Build history of the part. All positions in model axes, mm. Round coordinates to 2 decimals unless told otherwise and drop trailing zeros. Put each result on its own line as item: value. Start each with the question number.
Item 1: Drill centre lines: probe 1 along Y at (x, z) = (165, -16); probe 2 along Z at (x, y) = (-309.5, 5); probe 3 along Z at (x, y) = (425, -15). Where is each one in solid material? Low to high. Write a range as [from, to].
Item 2: Flat gauge pins, fed straight in: pin 1 Ø3 at (x, y) = (170.5, -19) entering from -Z; pin 2 Ø5 at (x, y) = (254, -0.5) entering from +Z; pin 3 Ø2 at (x, z) = (-299, 18.5) entering from -Y. Where does each tip first touch, or does it go through?
Item 3: Cut at A-A, the plane x = -300. Count the separate pieces of the cut face and the enclosed holes in it, plus the area to 3 significant figures.
```python
from build123d import *

# Parameters (mm, degrees)
SKETCH1_R                 = 3.4
SKETCH1_R_2               = 3
F_40_X_40W_X_R4_5_1_DEPTH = 1200


with BuildPart() as part:
    # Sketch1 → 铝型材 40 X 40W X R4.5(1) (new body)
    with BuildSketch(Plane(origin=(-600, 0, 0), x_dir=(0, 0, -1), z_dir=(1, 0, 0))):
        with BuildLine():
            Line((-5.1, 20), (-5.1, 19.5))
            Line((-5.1, 19.5), (-4.1, 19.5))
            Line((-4.1, 19.5), (-4.1, 17))
            Line((-4.1, 17), (-6.1, 17))
            Line((-6.1, 17), (-6.1, 18))
            Line((-6.1, 18), (-10.3, 18))
            Line((-10.3, 18), (-10.3, 12))
            Line((-10.3, 12), (-6, 7.7))
            Line((-6, 7.7), (6, 7.7))
            Line((6, 7.7), (10.3, 12))
            Line((10.3, 12), (10.3, 18))
            Line((10.3, 18), (6.1, 18))
            Line((6.1, 18), (6.1, 17))
            Line((6.1, 17), (4.1, 17))
            Line((4.1, 17), (4.1, 19.5))
            Line((4.1, 19.5), (5.1, 19.5))
            Line((5.1, 19.5), (5.1, 20))
            Line((5.1, 20), (15.5, 20))
            ThreePointArc((15.5, 20), (18.681980515, 18.681980515), (20, 15.5))
            Line((20, 15.5), (20, 5.1))
            Line((20, 5.1), (19.5, 5.1))
            Line((19.5, 5.1), (19.5, 4.1))
            Line((19.5, 4.1), (17, 4.1))
            Line((17, 4.1), (17, 6.1))
            Line((17, 6.1), (18, 6.1))
            Line((18, 6.1), (18, 10.3))
            Line((18, 10.3), (12, 10.3))
            Line((12, 10.3), (7.7, 6))
            Line((7.7, 6), (7.7, -6))
            Line((7.7, -6), (12, -10.3))
            Line((12, -10.3), (18, -10.3))
            Line((18, -10.3), (18, -6.1))
            Line((18, -6.1), (17, -6.1))
            Line((17, -6.1), (17, -4.1))
            Line((17, -4.1), (19.5, -4.1))
            Line((19.5, -4.1), (19.5, -5.1))
            Line((19.5, -5.1), (20, -5.1))
            Line((20, -5.1), (20, -15.5))
            ThreePointArc((20, -15.5), (18.681980515, -18.681980515), (15.5, -20))
            Line((15.5, -20), (5.1, -20))
            Line((5.1, -20), (5.1, -19.5))
            Line((5.1, -19.5), (4.1, -19.5))
            Line((4.1, -19.5), (4.1, -17))
            Line((4.1, -17), (6.1, -17))
            Line((6.1, -17), (6.1, -18))
            Line((6.1, -18), (10.3, -18))
            Line((10.3, -18), (10.3, -12))
            Line((10.3, -12), (6, -7.7))
            Line((6, -7.7), (-6, -7.7))
            Line((-6, -7.7), (-10.3, -12))
            Line((-10.3, -12), (-10.3, -18))
            Line((-10.3, -18), (-6.1, -18))
            Line((-6.1, -18), (-6.1, -17))
            Line((-6.1, -17), (-4.1, -17))
            Line((-4.1, -17), (-4.1, -19.5))
            Line((-4.1, -19.5), (-5.1, -19.5))
            Line((-5.1, -19.5), (-5.1, -20))
            Line((-5.1, -20), (-15.5, -20))
            ThreePointArc((-15.5, -20), (-18.681980515, -18.681980515), (-20, -15.5))
            Line((-20, -15.5), (-20, -5.1))
            Line((-20, -5.1), (-19.5, -5.1))
            Line((-19.5, -5.1), (-19.5, -4.1))
            Line((-19.5, -4.1), (-17, -4.1))
            Line((-17, -4.1), (-17, -6.1))
            Line((-17, -6.1), (-18, -6.1))
            Line((-18, -6.1), (-18, -10.3))
            Line((-18, -10.3), (-12, -10.3))
            Line((-12, -10.3), (-7.7, -6))
            Line((-7.7, -6), (-7.7, 6))
            Line((-7.7, 6), (-12, 10.3))
            Line((-12, 10.3), (-18, 10.3))
            Line((-18, 10.3), (-18, 6.1))
            Line((-18, 6.1), (-17, 6.1))
            Line((-17, 6.1), (-17, 4.1))
            Line((-17, 4.1), (-19.5, 4.1))
            Line((-19.5, 4.1), (-19.5, 5.1))
            Line((-19.5, 5.1), (-20, 5.1))
            Line((-20, 5.1), (-20, 15.5))
            ThreePointArc((-20, 15.5), (-18.681980515, 18.681980515), (-15.5, 20))
            Line((-15.5, 20), (-5.1, 20))
        make_face()
        Circle(SKETCH1_R, mode=Mode.SUBTRACT)
        with Locations((-15.556349186, 15.556349186)):
            Circle(SKETCH1_R_2, mode=Mode.SUBTRACT)
        with Locations((15.556349186, 15.556349186)):
            Circle(SKETCH1_R_2, mode=Mode.SUBTRACT)
        with Locations((15.556349186, -15.556349186)):
            Circle(SKETCH1_R_2, mode=Mode.SUBTRACT)
        with Locations((-15.556349186, -15.556349186)):
            Circle(SKETCH1_R_2, mode=Mode.SUBTRACT)
    extrude(amount=F_40_X_40W_X_R4_5_1_DEPTH)


solid = part.part
```
Reply:
1. probe 1: y = [-19.97, -18.52], [-12.59, -10.3], [10.3, 12.59], [18.52, 19.97]
1. probe 2: z = [-19.5, -17], [-7.7, 7.7], [17, 19.5]
1. probe 3: z = [-20, -18.5], [-12.61, -10.3], [10.3, 12.61], [18.5, 20]
2. pin 1: stops at z = -19.53
2. pin 2: stops at z = 7.7
2. pin 3: stops at y = -19.53
3. separate pieces: 1
3. enclosed holes: 5
3. area: 605 mm^2
